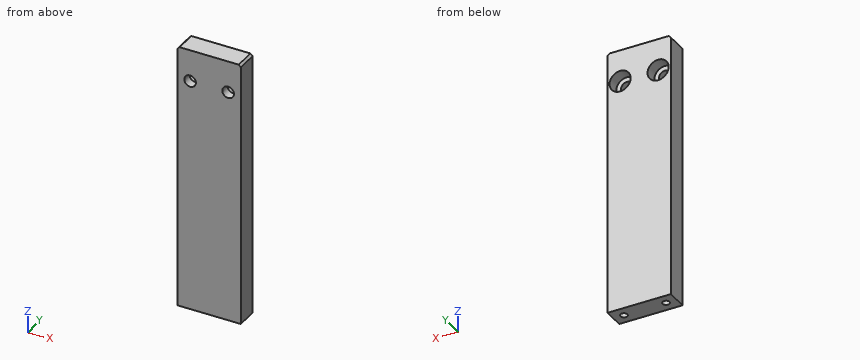
```python
from build123d import *

# Parameters (mm, degrees)
SKETCH_1_W                = 30
SKETCH_1_H                = 126
EXTRUDE_1_DEPTH           = 5
HOLE_WIZARD_1_D           = 5.5
HOLE_WIZARD_1_CBORE_D     = 10
HOLE_WIZARD_1_CBORE_DEPTH = 5.7
CHAMFER_1_SIZE            = 1
HOLE_WIZARD_M4_1_D        = 3.3
HOLE_WIZARD_M4_1_DEPTH    = 10.1
HOLE_WIZARD_M4_1_TIP      = 0.991420021


with BuildPart() as part:
    # 草图1 → 凸台-拉伸1 (new, symmetric)
    with BuildSketch(Plane(origin=(0, 0, 0), x_dir=(1, 0, 0), z_dir=(0, 1, 0))):
        Rectangle(SKETCH_1_W, SKETCH_1_H)
    extrude(amount=EXTRUDE_1_DEPTH, both=True)

    # 打孔尺寸(%根据)内六角圆柱头螺钉的类型1 (through all)
    with Locations(Plane(origin=(0, 5, 0), x_dir=(1, 0, 0), z_dir=(0, 1, 0))):
        with Locations((9, -48), (-9, -48)):
            CounterBoreHole(HOLE_WIZARD_1_D / 2, HOLE_WIZARD_1_CBORE_D / 2, HOLE_WIZARD_1_CBORE_DEPTH)

    # 倒角1
    chamfer_1_edges = [part.edges().sort_by_distance(p)[0] for p in [
        (15, 0, 63),
        (-15, 0, 63),
    ]]
    chamfer(chamfer_1_edges, length=CHAMFER_1_SIZE)

    # M4 螺纹孔1
    with Locations(Plane(origin=(0, 0, -63), x_dir=(-1, 0, 0), z_dir=(0, 0, -1))):
        with Locations((-10, 0), (10, 0)):
            Hole(HOLE_WIZARD_M4_1_D / 2, depth=HOLE_WIZARD_M4_1_DEPTH)
            with Locations((0, 0, -(HOLE_WIZARD_M4_1_DEPTH + HOLE_WIZARD_M4_1_TIP / 2))):  # 118° drill point
                Cone(0, HOLE_WIZARD_M4_1_D / 2, HOLE_WIZARD_M4_1_TIP, mode=Mode.SUBTRACT)


solid = part.part
```
Work out the finished part from the listing and answer in its coordinate system (mm). Give positions to 0.01 mm unless a question says otherwise; leave off trailing zeros. Write each loop counter-clockwise with the first axis right and the second up, starting at its lowest first coordinate (ties: lowest second). Pieces come first, ordered by that corner, then holes. Notation, with made-up numbers: (85.5, 61.25) - (91.5, 61.25) arc R21 cw to (91.5, 72.25) - close; hole circle Ø5 at (49.25, 30.25). An arc over 180 degrees is marked (long way). Use one line per item in the form item = value.
1. Consider L1, parallel to X at y = 0, z = -60.5; L2, parallel to X at y = -2.65, z = 48; L3, parallel to Z at x = -9, y = 2.05. Determine where each line is inside the solid, lowest interval first.
Filled in:
L1 = -15 to -11.65, -8.35 to 8.35, 11.65 to 15
L2 = -15 to -11.75, -6.25 to 6.25, 11.75 to 15
L3 = -63 to 43, 53 to 63
2. A cutting plane is placed at A-A (z = 48). Write down the section's boundary in (x, y), and give its area (3 significant figures).
Filled in:
outline = (-15, -5) - (-11.75, -5) - (-11.75, -0.7) - (-14, -0.7) - (-14, 5) - (-15, 5) - close; (-6.25, -5) - (6.25, -5) - (6.25, -0.7) - (4, -0.7) - (4, 5) - (-4, 5) - (-4, -0.7) - (-6.25, -0.7) - close; (11.75, -5) - (15, -5) - (15, 5) - (14, 5) - (14, -0.7) - (11.75, -0.7) - close
area = 139 mm^2
3. A cutting plane is placed at B-B (y = 3.5). Write down the section's boundary in (x, z), and give its area (3 significant figures).
Filled in:
outline = (-15, -63) - (15, -63) - (15, 62) - (14, 63) - (-14, 63) - (-15, 62) - close; hole circle Ø10 at (-9, 48); hole circle Ø10 at (9, 48)
area = 3,620 mm^2
4. Each of these flat-tipped pins is pushed along its axis until it touches: pin 1 Ø6 at (x, z) = (9, 48) entering from +Y; pin 2 Ø4.5 at (x, z) = (9, 48) entering from -Y; pin 3 Ø11 at (x, z) = (-8.5, 50) entering from +Y. Where does it stop, or does it pass through?
Filled in:
pin_1 = -0.7
pin_2 = through
pin_3 = 5
